The model under review builds one solid part; all positions refer to its coordinate system, in mm. Round coordinates to 2 decimals unless told otherwise and drop trailing zeros. Loops run counter-clockwise (first coordinate to the right, second up) from the corner with the lowest first, then second, coordinate; pieces in that order, holes last. Notation, with made-up numbers: M 11.25,36 L 53.25,36 A35 ccw 53.25,68 Z; hole C -29.75,11.25 d3. An arc over 180 degrees is marked long. Answer as a JSON object with one key per item and string values. Group by question number.
Item 1: Consider section B-B (y = 189.5). Give the boundary of the cut face in (x, z), and give its area (3 significant figures).
Item 2: To check wall thickness, follow line 1 (Y direction, x = 87, z = 3); line 2 (Y direction, x = 87.5, z = 1); line 3 (Y direction, x = 6, z = 6). State the ranges of each line that lie inside material, in increasing order.
Item 3: Insertion check: P1, Ø1.5, axis at y = 167.5, z = 6.5, coming from the +X side; P2, Ø3, axis at y = 117, z = 2.5, coming from the -X side; P3, Ø4, axis at x = 27, z = 6.5, coming from the -Y side. Each pin has a flat end and moves straight along its axis. Give the tip position at first contact, or say it passes through.
Item 4: Consider section A-A (z = 3). State how many separate pieces and enclosed holes the cut face has, and give its area (3 significant figures).
Item 5: Consider section C-C (x = 68). Give the boundary of the cut face in (y, z), and give its area (3 significant figures).
```python
from build123d import *

# Parameters (mm, degrees)
SKETCH_1_R          = 4.191
SKETCH_1_R_2        = 4.2
EXTRUDE_1_DEPTH     = 8
SKETCH_2_R          = 4
CUT_EXTRUDE_1_DEPTH = 20


with BuildPart() as part:
    # 草图1 → 凸台-拉伸1 (new body)
    with BuildSketch(Plane.XY):
        with BuildLine():
            Line((87.979357684, 127.610653672), (-1.529435027, 92.60618121))
            ThreePointArc((-1.529435027, 92.60618121), (-8.81810924, 92.751332474), (-13.869342758, 98.007840879))
            Line((-13.869342758, 98.007840879), (-19.159529273, 111.53520395))
            ThreePointArc((-19.159529273, 111.53520395), (-19.083334383, 115.361279652), (-16.324012386, 118.012845804))
            Line((-16.324012386, 118.012845804), (70.420477634, 151.936274108))
            ThreePointArc((70.420477634, 151.936274108), (70.975789492, 152.193666623), (71.49549165, 152.516980454))
            Line((71.49549165, 152.516980454), (137.996231332, 199.768508694))
            ThreePointArc((137.996231332, 199.768508694), (141.726549955, 200.622548455), (144.968180855, 198.588712168))
            Line((144.968180855, 198.588712168), (156.55248685, 182.285220069))
            ThreePointArc((156.55248685, 182.285220069), (157.406526611, 178.554901446), (155.372690324, 175.313270545))
            Line((155.372690324, 175.313270545), (89.054371699, 128.191360017))
            ThreePointArc((89.054371699, 128.191360017), (88.534669542, 127.868046187), (87.979357684, 127.610653672))
        make_face()
        with Locations((43.76834518, 120.548384653)):
            Circle(SKETCH_1_R, mode=Mode.SUBTRACT)
        with Locations((-4.998559058, 101.47696491)):
            Circle(SKETCH_1_R_2, mode=Mode.SUBTRACT)
    extrude(amount=EXTRUDE_1_DEPTH)

    # 草图2 → 切除-拉伸1 (cut)
    with BuildSketch(Plane.XY.offset(8)):
        with Locations((145.504664302, 180.568940096)):
            Circle(SKETCH_2_R)
        with Locations((88.422593517, 140.051817853)):
            Circle(SKETCH_2_R)
    extrude(amount=-CUT_EXTRUDE_1_DEPTH, mode=Mode.SUBTRACT)


solid = part.part
```
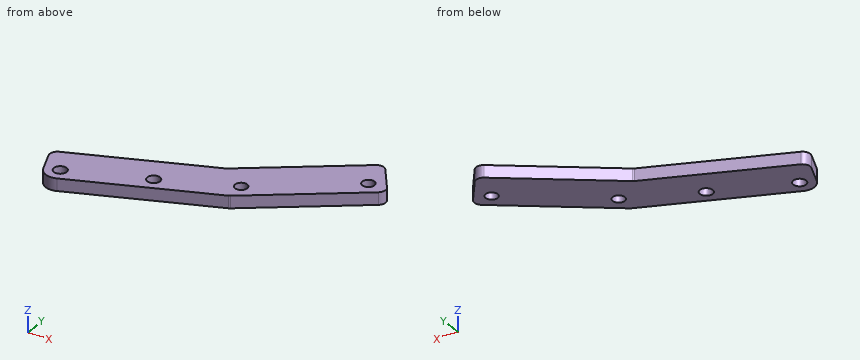
Geometry results:
{
 "1": {"outline": "M 123.54,0 L 151.43,0 L 151.43,8 L 123.54,8 Z", "area": "223 mm^2"},
 "2": {"line 1": "y = 127.23 to 136.31, 143.79 to 163.53", "line 2": "y = 127.42 to 136.16, 143.94 to 163.89", "line 3": "y = 95.55 to 126.74"},
 "3": {"P1": "stops at x = 145.43", "P2": "stops at x = -19.02", "P3": "stops at y = 102.98"},
 "4": {"separate pieces": "1", "enclosed holes": "4", "area": "5,340 mm^2"},
 "5": {"outline": "M 119.8,0 L 150.99,0 L 150.99,8 L 119.8,8 Z", "area": "250 mm^2"}
}
